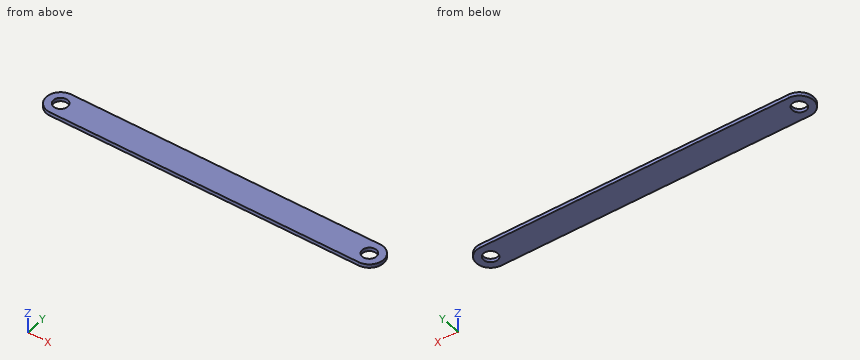
from build123d import *

# Parameters (mm, degrees)
SKETCH1_R           = 5
BOSS_EXTRUDE1_DEPTH = 2.5


with BuildPart() as part:
    # Sketch1 → Boss-Extrude1 (new body)
    with BuildSketch(Plane.XY):
        with BuildLine():
            Line((-110, 10), (110, 10))
            ThreePointArc((110, 10), (120, 0), (110, -10))
            Line((110, -10), (-110, -10))
            ThreePointArc((-110, -10), (-120, 0), (-110, 10))
        make_face()
        with Locations((-110, 0)):
            Circle(SKETCH1_R, mode=Mode.SUBTRACT)
        with Locations((110, 0)):
            Circle(SKETCH1_R, mode=Mode.SUBTRACT)
    extrude(amount=BOSS_EXTRUDE1_DEPTH)


solid = part.part
The model under review builds one solid part; all positions refer to its coordinate system, in mm. Round coordinates to 2 decimals unless told otherwise and drop trailing zeros. Loops run counter-clockwise (first coordinate to the right, second up) from the corner with the lowest first, then second, coordinate; pieces in that order, holes last. Notation, with made-up numbers: (88.25, 38.25) - (97.25, 38.25) arc R19 ccw to (97.25, 48.25) - close; hole circle Ø4 at (9, 55.25). An arc over 180 degrees is marked (long way). Use CSV: the item, a comma, the result in double quotes.
(1) For line 1 (Y direction, x = 110, z = 1.7); line 2 (X direction, y = -2, z = 1.25); line 3 (X direction, y = -4.5, z = 1.5), list the stretches that pass through material, from the lowest coordinate up.
Working result:
line 1,"y = -10 to -5, 5 to 10"
line 2,"x = -119.8 to -114.58, -105.42 to 105.42, 114.58 to 119.8"
line 3,"x = -118.93 to -112.18, -107.82 to 107.82, 112.18 to 118.93"
(2) Take a section at A-A, the plane y = 0. Give the boundary of the cut face in (x, z), plus the area to 3 significant figures.
Working result:
outline,"(-120, 0) - (-115, 0) - (-115, 2.5) - (-120, 2.5) - close; (-105, 0) - (105, 0) - (105, 2.5) - (-105, 2.5) - close; (115, 0) - (120, 0) - (120, 2.5) - (115, 2.5) - close"
area,"550 mm^2"
(3) Clearance check with flat-ended pins moving along their axes: P1, Ø6, axis at x = 110, y = 0, coming from the +Z side; P2, Ø1.5, axis at y = -6.5, z = 1.5, coming from the -X side. State where each tip first meets the part, or that it passes through.
Working result:
P1,"passes through"
P2,"stops at x = -118.18"
(4) Take a section at B-B, the plane z = 2. Give the boundary of the cut face in (x, y), plus the area to 3 significant figures.
Working result:
outline,"(-110, -10) - (110, -10) arc R10 ccw to (110, 10) - (-110, 10) arc R10 ccw to start; hole circle Ø10 at (-110, 0); hole circle Ø10 at (110, 0)"
area,"4,560 mm^2"
